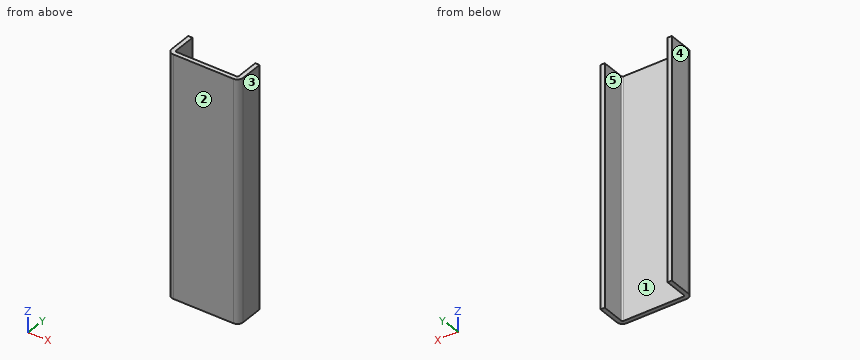
```python
from build123d import *

# Parameters (mm, degrees)
BOSS_EXTRUDE2_DEPTH = 337.5


with BuildPart() as part:
    # Sketch2 → Boss-Extrude2 (new body)
    with BuildSketch(Plane.XY):
        with BuildLine():
            Line((0, 0), (0, -32))
            ThreePointArc((0, -32), (2.343145751, -37.656854249), (8, -40))
            Line((8, -40), (92, -40))
            ThreePointArc((92, -40), (97.656854249, -37.656854249), (100, -32))
            Line((100, -32), (100, 0))
            Line((100, 0), (94, 0))
            Line((94, 0), (94, -32))
            ThreePointArc((94, -32), (93.414213562, -33.414213562), (92, -34))
            Line((92, -34), (8, -34))
            ThreePointArc((8, -34), (6.585786438, -33.414213562), (6, -32))
            Line((6, -32), (6, 0))
            Line((6, 0), (0, 0))
        make_face()
    extrude(amount=BOSS_EXTRUDE2_DEPTH)


solid = part.part
```
The model under review builds one solid part; all positions refer to its coordinate system, in mm. Face numbers are marked on the shaded views. A direction names the side the tool comes from. Coordinates: 2 decimals unless noted, no trailing zeros. Order: outer loops, then holes, each group sorted by start corner. A loop starts at its lowest first (then second) coordinate and runs counter-clockwise, first axis right, second up. Notation, with made-up numbers: M 46,83 L 102,83 A10 cw 102,102 Z; hole C -28.75,-12 d4. An arc over 180 degrees is marked long. One line per question, with ' | ' between items.
(1) Insertion check: pin 1 (5 mm diameter, centred on x = 62, z = 137.5, fed in from +Y). The pin has a flat end and moves straight along its axis. Give the tip position at first contact, or say it passes through.
Geometry results:
pin 1: stops at y = -34
(2) Add section C-C, the plane x = 64. Write out the cut boundary in (y, z), then the cut area to 4 significant figures.
Geometry results:
outline: M -40,0 L -34,0 L -34,337.5 L -40,337.5 Z | area: 2,025 mm²
(3) For probe 1 along X at (y, z) = (-11, 159); probe 2 along Y at (x, z) = (80.5, 238.5); probe 3 along X at (y, z) = (-36, 155.5), list the stretches that pass through material, from the lowest coordinate up. Write a range as from..to.
Geometry results:
probe 1: x = 0..6, 94..100 | probe 2: y = -40..-34 | probe 3: x = 1.07..98.93
(4) Add section A-A, the plane y = -20. Write out the cut boundary in (x, z).
Geometry results:
outline: M 0,0 L 6,0 L 6,337.5 L 0,337.5 Z; M 94,0 L 100,0 L 100,337.5 L 94,337.5 Z
(5) Machinability: for the marked faces 4 and 5, which of the approach directions +Z, -Z, +X, -X, +Y, -Y give a long, thin tool a straight path to every point of the face, cutting with its end or side? Answer none if there is none.
Geometry results:
face 4: +Z, -Z, -X, +Y, -Y | face 5: +Z, -Z, +Y
(6) Add section B-B, the plane z = 232.5. Write out the cut boundary in (x, y), then the cut area to 3 significant figures.
Geometry results:
outline: M 0,-32 A8 ccw 8,-40 L 92,-40 A8 ccw 100,-32 L 100,0 L 94,0 L 94,-32 A2 cw 92,-34 L 8,-34 A2 cw 6,-32 L 6,0 L 0,0 Z | area: 982 mm²
(7) The part is to be moulded in two halves that separate along X. For the marked faces 1, 2 and 3, say which applies: +X half, -X half, draft (parallel to the pull), parting line (faces both ways), or undercut.
Geometry results:
face 1: undercut | face 2: draft | face 3: +X half
